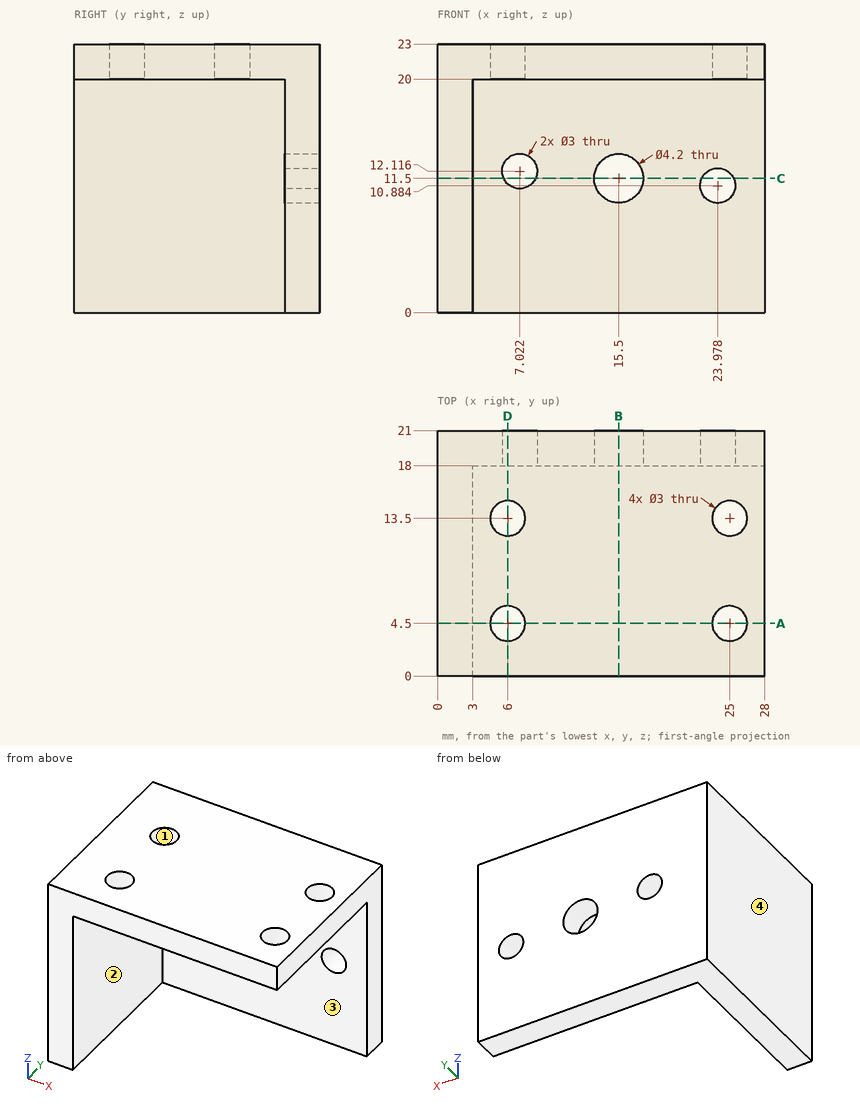
Can you work these out from the drawing? Everything is in mm from the part's minimum corner. Give positions to 0.01 mm unless a question says otherwise; leave off trailing zeros. Loops run counter-clockwise (first coordinate to the right, second up) from the corner with the lowest first, then second, coordinate; pieces in that order, holes last. Notation, with made-up numbers: (47, -5.75) -> (90, -5.75) arc R24 cw to (90, 27.25) -> close; hole circle Ø9 at (-37.75, 83.25). An arc over 180 degrees is marked (long way). Return JSON: item names as keys, results as strings.
Q1. I want a section at A-A, the plane y = 4.5. List the corners of the cut face in (x, z) for me, then the cut area to 3 significant figures.
Checks:
{"outline": "(0, 0) -> (3, 0) -> (3, 20) -> (4.5, 20) -> (4.5, 23) -> (0, 23) -> close; (7.5, 20) -> (23.5, 20) -> (23.5, 23) -> (7.5, 23) -> close; (26.5, 20) -> (28, 20) -> (28, 23) -> (26.5, 23) -> close", "area": "126 mm2"}
Q2. I want a section at B-B, the plane x = 15.5. List the corners of the cut face in (y, z) for me, then the cut area to 3 significant figures.
Checks:
{"outline": "(0, 20) -> (18, 20) -> (18, 13.6) -> (21, 13.6) -> (21, 23) -> (0, 23) -> close; (18, 0) -> (21, 0) -> (21, 9.4) -> (18, 9.4) -> close", "area": "110 mm2"}
Q3. I want a section at D-D, the plane x = 6. List the corners of the cut face in (y, z) for me.
Checks:
{"outline": "(0, 20) -> (3, 20) -> (3, 23) -> (0, 23) -> close; (6, 20) -> (12, 20) -> (12, 23) -> (6, 23) -> close; (15, 20) -> (18, 20) -> (18, 13.21) -> (21, 13.21) -> (21, 23) -> (15, 23) -> close; (18, 0) -> (21, 0) -> (21, 11.02) -> (18, 11.02) -> close"}
Q4. We'd pull the mould along X, two halves only. Please class the marked faces 1, 2, 3 and 4: released by +X, released by -X, zero draft, split by the parting line, or undercut.
Checks:
{"face 1": "undercut", "face 2": "released by +X", "face 3": "zero draft", "face 4": "released by -X"}
Q5. I need wall thicknesses on probe 1 along Y at (x, z) = (6, 22.25); probe 2 along X at (y, z) = (18.75, 10.75) (1 decimal); probe 3 along Z at (x, y) = (25.5, 17.5). Which ranges of each line are inside material? Lowest first, please.
Checks:
{"probe 1": "y = 0 to 3, 6 to 12, 15 to 21", "probe 2": "x = 0 to 6.4, 7.6 to 13.5, 17.5 to 22.5, 25.5 to 28", "probe 3": "z = 20 to 23"}
Q6. For pin 1 Ø5 at (x, y) = (6, 13.5) entering from +Z; pin 2 Ø5.5 at (x, y) = (19, 8.5) entering from -Z; pin 3 Ø5.5 at (y, z) = (7, 9.5) entering from +X; pin 4 Ø3 at (x, z) = (22, 12.5) entering from -Y, each with a flat end and sliding along its axis, tell me the tip position at first contact or that it passes through.
Checks:
{"pin 1": "stops at z = 23", "pin 2": "stops at z = 20", "pin 3": "stops at x = 3", "pin 4": "stops at y = 18"}
Q7. I want a section at C-C, the plane z = 11.5. List the corners of the cut face in (x, y) for me (1 decimal).
Checks:
{"outline": "(0, 0) -> (3, 0) -> (3, 18) -> (5.7, 18) -> (5.7, 21) -> (0, 21) -> close; (8.4, 18) -> (13.4, 18) -> (13.4, 21) -> (8.4, 21) -> close; (17.6, 18) -> (22.6, 18) -> (22.6, 21) -> (17.6, 21) -> close; (25.3, 18) -> (28, 18) -> (28, 21) -> (25.3, 21) -> close"}
